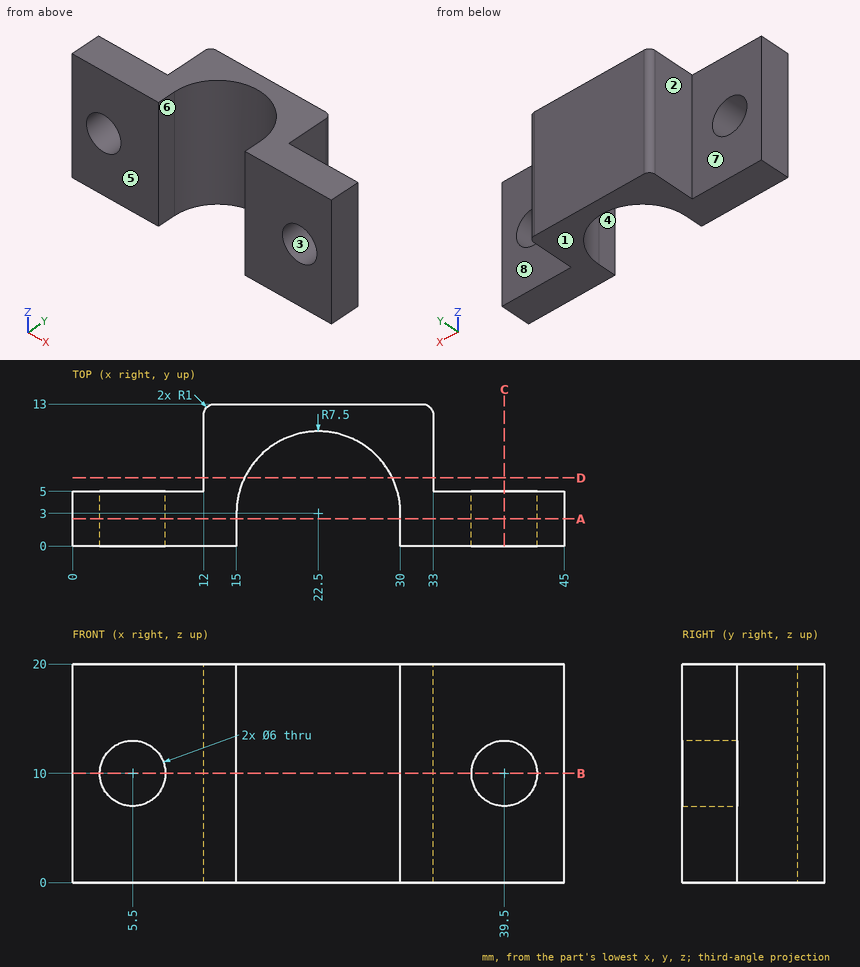
Drawing for the job (mm, zero at the part's lowest x, y, z). A direction names the side the tool comes from. Give positions to 0.01 mm unless a question says otherwise; leave off trailing zeros. Loops run counter-clockwise (first coordinate to the right, second up) from the corner with the lowest first, then second, coordinate; pieces in that order, holes last.
1) Band-saw the part on C-C on x = 39.5. List the corners of the cut face in (y, z), then the cut area to 3 significant figures.
Values follow:
outline: (0, 0) - (5, 0) - (5, 7) - (0, 7) - close; (0, 13) - (5, 13) - (5, 20) - (0, 20) - close
area: 70.0 mm2
2) Band-saw the part on B-B on z = 10. List the corners of the cut face in (x, y), then the cut area to 3 significant figures.
Values follow:
outline: (0, 0) - (2.5, 0) - (2.5, 5) - (0, 5) - close; (8.5, 0) - (15, 0) - (15, 3) arc R7.5 cw to (30, 3) - (30, 0) - (36.5, 0) - (36.5, 5) - (33, 5) - (33, 12) arc R1 ccw to (32, 13) - (13, 13) arc R1 ccw to (12, 12) - (12, 5) - (8.5, 5) - close; (42.5, 0) - (45, 0) - (45, 5) - (42.5, 5) - close
area: 199 mm2
3) Band-saw the part on A-A on y = 2.5. List the corners of the cut face in (x, z).
Values follow:
outline: (0, 0) - (15, 0) - (15, 20) - (0, 20) - close; (30, 0) - (45, 0) - (45, 20) - (30, 20) - close; hole circle Ø6 at (5.5, 10); hole circle Ø6 at (39.5, 10)
4) Drop flat-ended pins along their axis: P1, Ø5, axis at x = 39, z = 11.5, coming from the +Y side; P2, Ø1, axis at x = 17.5, y = 3, coming from the +Z side; P3, Ø5.5, axis at y = 9, z = 5, coming from the +X side. Give the stop position or say it passes through.
Values follow:
P1: stops at y = 5
P2: passes through
P3: stops at x = 33
5) Band-saw the part on D-D on y = 6.25. List the corners of the cut face in (x, z), then the cut area to 3 significant figures.
Values follow:
outline: (12, 0) - (15.74, 0) - (15.74, 20) - (12, 20) - close; (29.26, 0) - (33, 0) - (33, 20) - (29.26, 20) - close
area: 150 mm2
6) Two-plate mould, pull along X, no slides. Class the marked faces 1, 2, 3 and 4: released by +X, released by -X, zero draft, split by the parting line, or undercut.
Values follow:
face 1: zero draft
face 2: released by -X
face 3: undercut
face 4: undercut
7) 3-axis set-ups, long thin cutter, end or side, ignore diameter. For the marked faces 5, 6, 7 and 8: which of +Z, -Z, +X, -X, +Y, -Y reach the whole face in a straight line?
Values follow:
face 5: +Z, -Z, +X, -X, -Y
face 6: +Z, -Z, -Y
face 7: +Z, -Z, -X, +Y
face 8: +Z, -Z, +X, +Y
8) Probe line 1 along X through (y, z) = (1.25, 10); line 2 along X through (y, z) = (1.5, 14); line 3 along Z through (x, y) = (37, 3.75). List the from-to ranges inside material, lowest first.
Values follow:
line 1: x = 0 to 2.5, 8.5 to 15, 30 to 36.5, 42.5 to 45
line 2: x = 0 to 15, 30 to 45
line 3: z = 0 to 8.34, 11.66 to 20
